from build123d import *

# Parameters (mm, degrees)
SWEEP_1_PROFILE_R = 6


with BuildPart() as part:
    # 扫描1: sweep along a path in 草图1
    with BuildLine(Plane.XY) as sweep_1_path:
        Line((0, 0), (-67.781745931, 67.781745931))
        ThreePointArc((-67.781745931, 67.781745931), (-69.949473444, 71.025979419), (-70.710678119, 74.852813742))
        Line((-70.710678119, 74.852813742), (-70.710678119, 249.710678119))
        ThreePointArc((-70.710678119, 249.710678119), (-49.710678119, 270.710678119), (-28.710678119, 249.710678119))
        Line((-28.710678119, 249.710678119), (-28.710678119, 214.710678119))
    # 扫描1 profile (on start of the path) → 扫描1 (sweep)
    with BuildSketch(Plane(origin=(0, 0, 0), x_dir=(-0.7071067811865462, -0.7071067811865488, 0), z_dir=(-0.7071067811865488, 0.7071067811865462, 0))):
        Circle(SWEEP_1_PROFILE_R)
    sweep(path=sweep_1_path.line)


solid = part.part
Read the model definition and answer for the solid it produces. Units are mm, in the model's axes. A direction names the side the tool comes from. Give positions to 0.01 mm unless a question says otherwise; leave off trailing zeros. Write each loop counter-clockwise with the first axis right and the second up, starting at its lowest first coordinate (ties: lowest second). Pieces come first, ordered by that corner, then holes. Notation, with made-up numbers: (-19, 13) - (-13, 13) arc R19 ccw to (-13, 41) - close; hole circle Ø3 at (57, 2). An arc over 180 degrees is marked (long way). Answer in a Markdown table with one row per item. Add a question column.
Item 1: A tool of negligible diameter and unlimited length cuts with its end or side. For faces 3 (the face through (-29, 214.711, 0)), 4 (the face through (-34.705, 231.966, 0.264)), from which of +Z, -Z, +X, -X, +Y, -Y can it reach the whole face along a straight path? Write none if from no direction.
Item 2: Find the intervals of material crossed by L1, parallel to Y at x = -38, z = 3; L2, parallel to Z at x = -12.5, y = 13; L3, parallel to Y at x = -27.5, z = -4, in increasing order.
Item 3: Section B-B, the plane y = 154 is taken. Write down the section's boundary in (x, z), and give its area (3 significant figures).
Item 4: Determine the mould class of faces 1 (the face through (0, 0, 0)), 2 (the face through (-38, 30, 2)) for opening direction Y: pulls with the +Y half, pulls with the -Y half, needs draft (parallel to the pull), parting line crosses it, or undercut.
Item 5: Section A-A, the plane z = 0 is taken. Write down the section's boundary in (x, y).
Item 6: Flat-ended cylindrical pins translate along their axes: P1, Ø1.5, axis at x = -51, z = -2.5, coming from the -Y side; P2, Ø4, axis at y = 235, z = -4, coming from the +X side; P3, Ø5, axis at y = 187, z = 3, coming from the -X side; P4, Ø1, axis at x = -55, y = 67, coming from the -Z side. Find the tip coordinate at first contact, or state that the pin passes through.
Recorded:
| question | item | result |
|---|---|---|
| 1 | face 3 | +Z, -Z, +X |
| 1 | face 4 | none |
| 2 | L1 | y = 30.65 to 45.35, 260.32 to 273.14 |
| 2 | L2 | z = -5.99 to 5.99 |
| 2 | L3 | y = 21.18 to 33.82, 214.71 to 262.18 |
| 3 | outline | circle Ø12 at (-70.71, 0) |
| 3 | area | 113 mm2 |
| 4 | face 1 | pulls with the -Y half |
| 4 | face 2 | undercut |
| 5 | outline | (-76.71, 74.85) arc R16 ccw to (-72.02, 63.54) - (-4.24, -4.24) - (4.24, 4.24) - (-63.54, 72.02) arc R4 cw to (-64.71, 74.85) - (-64.71, 249.71) arc R15 cw to (-34.71, 249.71) - (-34.71, 214.71) - (-22.71, 214.71) - (-22.71, 249.71) arc R27 ccw to (-76.71, 249.71) - close |
| 6 | P1 | stops at y = 42.41 |
| 6 | P2 | stops at x = -23.05 |
| 6 | P3 | stops at x = -76.69 |
| 6 | P4 | passes through |
